```python
from build123d import *

# Parameters (mm, degrees)
BASE_EXTRUDE_DEPTH = 15
SKETCH4_W          = 0.8
SKETCH4_H          = 12.784609691
CHAMFER_2_SIZE     = 2.4
FILLET_2_R         = 0.8


with BuildPart() as part:
    # Sketch1 → Base-Extrude (new body)
    with BuildSketch(Plane(origin=(0, 0, 0), x_dir=(0, 0, -1), z_dir=(1, 0, 0))):
        Polygon((18, 10.392304845), (18, -10.392304845), (0, -20.784609691), (-18, -10.392304845), (-18, 10.392304845), (0, 20.784609691), align=None)
    extrude(amount=BASE_EXTRUDE_DEPTH)

    # Sketch2 → Boss-Revolve1 (revolve)
    with BuildSketch(Plane.XY, mode=Mode.PRIVATE) as boss_revolve1_sk:
        Polygon((0, 0), (200, 0), (200, 9.402), (200, 12), (27.8072, 12), (0, 12), align=None)
    revolve(boss_revolve1_sk.sketch.rotate(Axis((0, 0, 0), (1, 0, 0)), 90), axis=Axis((0, 0, 0), (1, 0, 0)))

    # Sketch3 → Cut-Revolve1 (revolve, cut)
    with BuildSketch(Plane.XY):
        Polygon((0, 18), (4.494446501, 25.784609691), (4.494446501, 30.784609691), (-10, 30.784609691), (-10, 18), align=None)
    revolve(axis=Axis((0, 0, 0), (1, 0, 0)), mode=Mode.SUBTRACT)

    # Sketch5 → Cut-Revolve2 (revolve, cut)
    with BuildSketch(Plane.XY):
        Polygon((15, 18), (10.505553499, 25.784609691), (10.505553499, 30.784609691), (20.505553499, 30.784609691), (20.505553499, 18), align=None)
    revolve(axis=Axis((0, 0, 0), (1, 0, 0)), mode=Mode.SUBTRACT)

    # Sketch4 → Cut-Revolve3 (revolve, cut)
    with BuildSketch(Plane.XY, mode=Mode.PRIVATE) as cut_revolve3_sk:
        with Locations((14.6, 24.392304845)):
            Rectangle(SKETCH4_W, SKETCH4_H)
    revolve(cut_revolve3_sk.sketch.rotate(Axis((0, 0, 0), (1, 0, 0)), 270), axis=Axis((0, 0, 0), (1, 0, 0)), mode=Mode.SUBTRACT)

    # Chamfer 2
    chamfer_2_edges = [part.edges().sort_by_distance(p)[0] for p in [
        (200, 0, -12),
    ]]
    chamfer(chamfer_2_edges, length=CHAMFER_2_SIZE)

    # Fillet 2
    fillet_2_edges = [part.edges().sort_by_distance(p)[0] for p in [
        (15, 0, -12),
    ]]
    fillet(fillet_2_edges, radius=FILLET_2_R)


solid = part.part
```
Geometry check sheet. Reference: the model listing, model coordinates, mm. A direction names the side the tool comes from. Give positions to 0.01 mm unless a question says otherwise; leave off trailing zeros. Order: outer loops, then holes, each group sorted by start corner. A loop starts at its lowest first (then second) coordinate and runs counter-clockwise, first axis right, second up. Notation, with made-up numbers: (18.5, 76.25) - (24.5, 76.25) arc R26 ccw to (24.5, 97.25) - close; hole circle Ø6 at (45, 60). An arc over 180 degrees is marked (long way). Answer in a Markdown table with one row per item. Add a question column.
Q1. Material ranges on probe 1 along X at (y, z) = (-17, -3.5); probe 2 along Z at (x, y) = (74, 0.5); probe 3 along Y at (x, z) = (190, -1), recorded low to high. Write a range as from..to.
Q2. Cross-section at A-A, the plane x = 46. Enter the section's corners in (y, z).
Q3. Tool access check on faces 1 (the flat face through (14.2, 18.2, 0)), 2 (the flat face through (14.2, 9, -16)), 3 (the cylindrical face through (14.606, -10.953, 14.284)). Record the directions out of +Z, -Z, +X, -X, +Y, -Y that give a thin tool (end or side, any length) a straight path to the whole face; none if there is none.
Q4. Gauge pin test, flat ends, axial feed: pin 1 (7 mm diameter, centred on y = 10.5, z = -13, fed in from +X); pin 2 (10 mm diameter, centred on y = 4.5, z = 13.5, fed in from +X); pin 3 (10 mm diameter, centred on y = -6, z = -15.5, fed in from +X); pin 4 (10 mm diameter, centred on y = -6, z = 15, fed in from +X). Record the tip position at first contact, or that the pin passes through.
Check values:
| question | item | result |
|---|---|---|
| 1 | probe 1 | x = 0..15 |
| 1 | probe 2 | z = -11.99..11.99 |
| 1 | probe 3 | y = -11.96..11.96 |
| 2 | outline | circle Ø24 at (0, 0) |
| 3 | face 1 | +X, +Y |
| 3 | face 2 | -Z, +X, +Y |
| 3 | face 3 | +X |
| 4 | pin 1 | stops at x = 15 |
| 4 | pin 2 | stops at x = 200 |
| 4 | pin 3 | stops at x = 197.98 |
| 4 | pin 4 | stops at x = 198.44 |
